Study the drawing (mm; zero at the part's minimum x, y, z) and answer. A direction names the side the tool comes from. Coordinates: 2 decimals unless noted, no trailing zeros. Order: outer loops, then holes, each group sorted by start corner. A loop starts at its lowest first (then second) coordinate and runs counter-clockwise, first axis right, second up. Notation, with made-up numbers: (66.25, 21.5) -> (90.25, 21.5) arc R32 cw to (90.25, 52.5) -> close; hole circle Ø9 at (18, 45.5). An arc over 180 degrees is marked (long way). Answer in a Markdown table with one row per item. Add a question column.
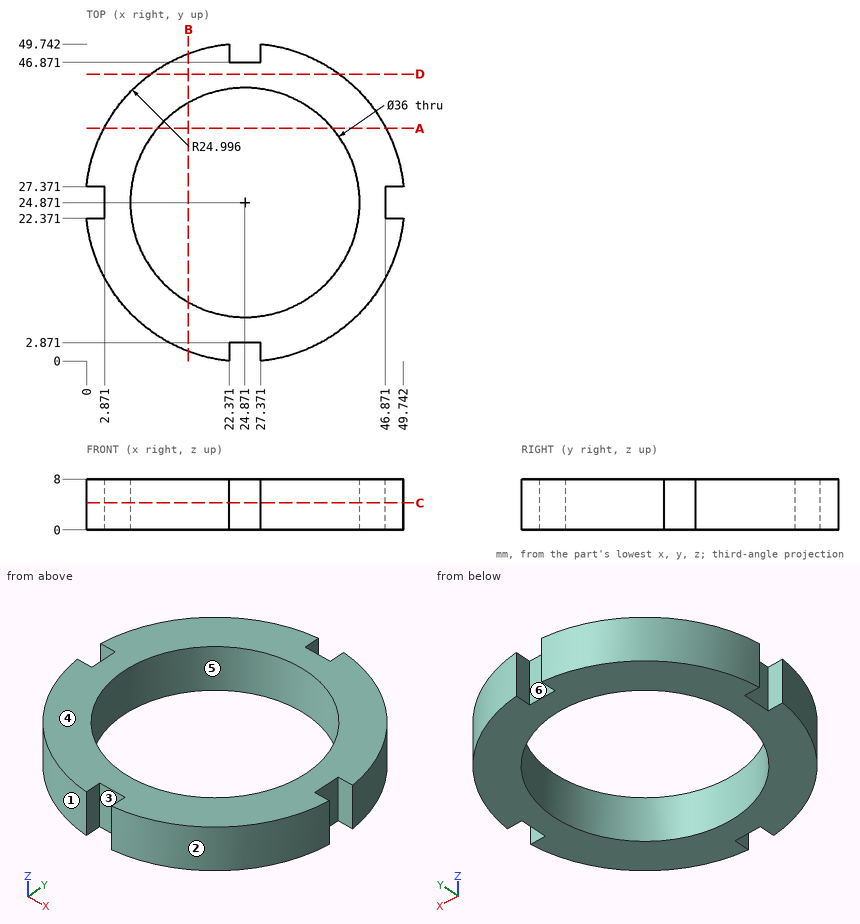
Q1. For the marked faces 5 and 6, determine the directions among +Z, -Z, +X, -X, +Y, -Y from which every point of the face is accessible in a straight line to the end or side of a thin tool.
Q2. A cutting plane is placed at B-B (x = 16). Determine the outline of the cut face in (y, z).
Q3. Given pin 1 (2.5 mm diameter, centred on y = 25, z = 4, fed in from +X); pin 2 (1.4 mm diameter, centred on x = 1.5, z = 4.5, fed in from +Y); pin 3 (1.5 mm diameter, centred on x = 25, z = 5.5, fed in from +Y), each flat-ended and moving along its own axis, determine where each tip first touches the part or whether it passes through.
Q4. A cutting plane is placed at D-D (y = 45). Determine the outline of the cut face in (x, z).
Q5. A cutting plane is placed at C-C (z = 4.25). Determine the outline of the cut face in (x, y).
Q6. Straight lines are drawn through the part: line 1 (X direction, y = 17, z = 1.25) (1 decimal); line 2 (Y direction, x = 23, z = 4.25); line 3 (X direction, y = 37.5, z = 3) (1 decimal). For each, find the intervals that lie inside material, in ascending order.
Q7. Determine the mould class of the marked faces 1, 2, 3 and 4 for opening direction X: +X half, -X half, draft (parallel to the pull), parting line (faces both ways), or undercut.
Q8. A cutting plane is placed at A-A (y = 36.5). Determine the outline of the cut face in (x, z) (1 decimal).
Returned:
| question | item | result |
|---|---|---|
| 1 | face 5 | +Z, -Z |
| 1 | face 6 | +Z, -Z, +Y |
| 2 | outline | (1.5, 0) -> (9.21, 0) -> (9.21, 8) -> (1.5, 8) -> close; (40.53, 0) -> (48.24, 0) -> (48.24, 8) -> (40.53, 8) -> close |
| 3 | pin 1 | stops at x = 46.87 |
| 3 | pin 2 | stops at y = 35.4 |
| 3 | pin 3 | stops at y = 46.87 |
| 4 | outline | (10.05, 0) -> (39.69, 0) -> (39.69, 8) -> (10.05, 8) -> close |
| 5 | outline | (0, 22.37) arc R25 ccw to (22.37, 0) -> (22.37, 2.87) -> (27.37, 2.87) -> (27.37, 0) arc R25 ccw to (49.74, 22.37) -> (46.87, 22.37) -> (46.87, 27.37) -> (49.74, 27.37) arc R25 ccw to (27.37, 49.74) -> (27.37, 46.87) -> (22.37, 46.87) -> (22.37, 49.74) arc R25 ccw to (0, 27.37) -> (2.87, 27.37) -> (2.87, 22.37) -> close; hole circle Ø36 at (24.87, 24.87) |
| 6 | line 1 | x = 1.1 to 8.7, 41.1 to 48.6 |
| 6 | line 2 | y = 2.87 to 6.97, 42.77 to 46.87 |
| 6 | line 3 | x = 3.3 to 12, 37.7 to 46.4 |
| 7 | face 1 | -X half |
| 7 | face 2 | +X half |
| 7 | face 3 | undercut |
| 7 | face 4 | draft |
| 8 | outline | (2.7, 0) -> (11.1, 0) -> (11.1, 8) -> (2.7, 8) -> close; (38.6, 0) -> (47, 0) -> (47, 8) -> (38.6, 8) -> close |
